```python
from build123d import *

# Parameters (mm, degrees)
BASE_DISC_SKETCH_R = 46
BASE_DISC_92_DEPTH = 3
RIM_START          = 9.5
RIM_SKETCH_R       = 46
RIM_SKETCH_R_2     = 40
RIM_92X_80_DEPTH   = 9.5
HUB_SKETCH_R       = 19
HUB_SKETCH_R_2     = 12.5
HUB_38_DEPTH       = 25
BORE_SKETCH_R      = 12.5
BORE_25_DEPTH      = 25


with BuildPart() as part:
    # Base Disc Sketch → Base Disc Ø92 (new, symmetric)
    with BuildSketch(Plane(origin=(0, 0, 0), x_dir=(1, 0, 0), z_dir=(0, 1, 0))):
        with Locations(Location((0, 0, 0), (0, 0, 270))):
            Circle(BASE_DISC_SKETCH_R)
    extrude(amount=BASE_DISC_92_DEPTH, both=True)

    # Rim Sketch → Rim Ø92xØ80 (add)
    with BuildSketch(Plane(origin=(0, 3, 0), x_dir=(1, 0, 0), z_dir=(0, 1, 0)).offset(RIM_START)):
        with Locations(Location((0, 0, 0), (0, 0, 270))):
            Circle(RIM_SKETCH_R)
        with Locations(Location((0, 0, 0), (0, 0, 270))):
            Circle(RIM_SKETCH_R_2, mode=Mode.SUBTRACT)
    rim_92x_80 = extrude(amount=-RIM_92X_80_DEPTH)

    # Rim Mirror: Rim Ø92xØ80 across plane
    add(rim_92x_80.mirror(Plane.ZX))

    # Hub Sketch → Hub Ø38 (add)
    with BuildSketch(Plane(origin=(0, 12.5, 0), x_dir=(1, 0, 0), z_dir=(0, 1, 0))):
        with Locations(Location((0, 0, 0), (0, 0, 270))):
            Circle(HUB_SKETCH_R)
        with Locations(Location((0, 0, 0), (0, 0, 270))):
            Circle(HUB_SKETCH_R_2, mode=Mode.SUBTRACT)
    extrude(amount=-HUB_38_DEPTH)

    # Bore Sketch → Bore Ø25 (cut)
    with BuildSketch(Plane(origin=(0, 3, 0), x_dir=(1, 0, 0), z_dir=(0, 1, 0))):
        with Locations(Location((0, 0, 0), (0, 0, 270))):
            Circle(BORE_SKETCH_R)
    extrude(amount=-BORE_25_DEPTH, mode=Mode.SUBTRACT)


solid = part.part
```
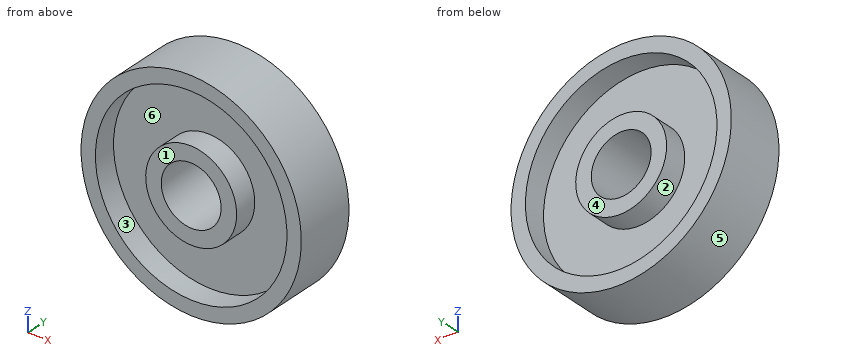
Check sheet for the modelled part. Datum: model origin and axes. Units: mm. Face numbers are marked on the shaded views. A direction names the side the tool comes from. Round coordinates to 2 decimals unless told otherwise and drop trailing zeros. Order: outer loops, then holes, each group sorted by start corner. A loop starts at its lowest first (then second) coordinate and runs counter-clockwise, first axis right, second up. Notation, with made-up numbers: M -16.5,48.5 L 16.5,48.5 A24 cw 16.5,82.5 Z; hole C -6.75,27 d5. An arc over 180 degrees is marked long. Answer in a Markdown table with one row per item.
(1) Section check D-D on y = 0.75. Record the boundary of the cut face in (x, z), plus the area to 3 significant figures.
Findings:
| item | result |
|---|---|
| outline | C 0,0 d92; hole C 0,0 d25 |
| area | 6,160 mm^2 |
(2) Draft check along X on the marked faces 4, 5 and 6. Enter one of: +X half, -X half, draft (parallel to the pull), parting line (faces both ways), or undercut.
Findings:
| item | result |
|---|---|
| face 4 | draft |
| face 5 | parting line |
| face 6 | undercut |
(3) Section check C-C on y = 8. Record the boundary of the cut face in (x, z).
Findings:
| item | result |
|---|---|
| outline | C 0,0 d92; C 0,0 d38; hole C 0,0 d80; hole C 0,0 d25 |
(4) Material ranges on line 1 along X through (y, z) = (-4.5, 0); line 2 along Z through (x, y) = (6, 4.5); line 3 along X through (y, z) = (1.75, 0), recorded low to high. Write a range as from..to.
Findings:
| item | result |
|---|---|
| line 1 | x = -46..-40, -19..-12.5, 12.5..19, 40..46 |
| line 2 | z = -45.61..-39.55, -18.03..-10.97, 10.97..18.03, 39.55..45.61 |
| line 3 | x = -46..-12.5, 12.5..46 |
(5) Section check A-A on z = 0. Record the boundary of the cut face in (x, y).
Findings:
| item | result |
|---|---|
| outline | M -46,-12.5 L -40,-12.5 L -40,-3 L -19,-3 L -19,-12.5 L -12.5,-12.5 L -12.5,12.5 L -19,12.5 L -19,3 L -40,3 L -40,12.5 L -46,12.5 Z; M 12.5,-12.5 L 19,-12.5 L 19,-3 L 40,-3 L 40,-12.5 L 46,-12.5 L 46,12.5 L 40,12.5 L 40,3 L 19,3 L 19,12.5 L 12.5,12.5 Z |
(6) Gauge pin test, flat ends, axial feed: pin 1 (2 mm diameter, centred on x = -23.5, y = -6.5, fed in from +Z); pin 2 (15 mm diameter, centred on x = 0, z = 0, fed in from -Y); pin 3 (5 mm diameter, centred on x = 18.5, y = 7, fed in from -Z); pin 4 (1 mm diameter, centred on x = 25, y = -6, fed in from -Z). Record the tip position at first contact, or that the pin passes through.
Findings:
| item | result |
|---|---|
| pin 1 | stops at z = 40.12 |
| pin 2 | passes through |
| pin 3 | stops at z = -43.13 |
| pin 4 | stops at z = -38.93 |
(7) Set-up check for the marked faces 1, 2 and 3: record each of +Z, -Z, +X, -X, +Y, -Y from which the full face is reachable in a straight line by a thin tool's end or side.
Findings:
| item | result |
|---|---|
| face 1 | +Z, -Z, +X, -X, -Y |
| face 2 | +Y |
| face 3 | -Y |
(8) Section check B-B on x = 0. Record the boundary of the cut face in (y, z), plus the area to 3 significant figures.
Findings:
| item | result |
|---|---|
| outline | M -12.5,-46 L 12.5,-46 L 12.5,-40 L 3,-40 L 3,-19 L 12.5,-19 L 12.5,-12.5 L -12.5,-12.5 L -12.5,-19 L -3,-19 L -3,-40 L -12.5,-40 Z; M -12.5,12.5 L 12.5,12.5 L 12.5,19 L 3,19 L 3,40 L 12.5,40 L 12.5,46 L -12.5,46 L -12.5,40 L -3,40 L -3,19 L -12.5,19 Z |
| area | 877 mm^2 |
